Could you check a few things on this model? Use its own coordinates, in mm. Give positions to 0.01 mm unless a question says otherwise; leave off trailing zeros. Write each loop counter-clockwise with the first axis right and the second up, starting at its lowest first coordinate (ties: lowest second). Pieces come first, ordered by that corner, then holes. Notation, with made-up numbers: M 75,19 L 80,19 A35 cw 80,54 Z; hole C 30.5,14.5 d2. An arc over 180 degrees is marked long. Use one line per item in the form item = value.
from build123d import *

# Parameters (mm, degrees)
SKETCH1_W           = 150
SKETCH1_H           = 80
BOSS_EXTRUDE1_DEPTH = 14
M8_TAPPED_HOLE1_D   = 6.8


with BuildPart() as part:
    # Sketch1 → Boss-Extrude1 (new body)
    with BuildSketch(Plane(origin=(0, 0, 0), x_dir=(1, 0, 0), z_dir=(0, 1, 0))):
        with Locations((75, 40)):
            Rectangle(SKETCH1_W, SKETCH1_H)
    extrude(amount=BOSS_EXTRUDE1_DEPTH)

    # M8 Tapped Hole1 (through all)
    with Locations(Plane(origin=(0, 14, 0), x_dir=(-1, 0, 0), z_dir=(0, 1, 0))):
        with Locations((-25, -65), (-25, -15), (-125, -15), (-125, -65)):
            Hole(M8_TAPPED_HOLE1_D / 2)


solid = part.part
1) Thinking about a two-plate mould opening in X: for faces 1 (the flat face through (0, 7, -39)), 2 (the flat face through (74, 14, -41)), 3 (the cylindrical face through (26.6, 6.9, -68)), which applies, released by +X, released by -X, zero draft, split by the parting line, or undercut?
Checked values:
face_1 = released by -X
face_2 = zero draft
face_3 = undercut
2) I want a section at B-B, the plane x = 25. Please give me the cut outline in (y, z), plus the area to 3 significant figures.
Checked values:
outline = M 0,-80 L 14,-80 L 14,-68.4 L 0,-68.4 Z; M 0,-61.6 L 14,-61.6 L 14,-18.4 L 0,-18.4 Z; M 0,-11.6 L 14,-11.6 L 14,0 L 0,0 Z
area = 930 mm2
3) I want a section at A-A, the plane z = -15. Please give me the cut outline in (x, y).
Checked values:
outline = M 0,0 L 21.6,0 L 21.6,14 L 0,14 Z; M 28.4,0 L 121.6,0 L 121.6,14 L 28.4,14 Z; M 128.4,0 L 150,0 L 150,14 L 128.4,14 Z
4) If I drill on L1, parallel to Z at x = 125, y = 10.75; L2, parallel to X at y = 1.75, z = -66.5, over which ranges is the centre line in solid material (lowest first)?
Checked values:
L1 = -80 to -68.4, -61.6 to -18.4, -11.6 to 0
L2 = 0 to 21.95, 28.05 to 121.95, 128.05 to 150
